```python
from build123d import *

# Parameters (mm, degrees)
SKETCH_1_W          = 58
SKETCH_1_H          = 62
EXTRUDE_1_DEPTH     = 10
SKETCH_2_W          = 46
SKETCH_2_H          = 62
CUT_EXTRUDE_1_DEPTH = 1.5
CHAMFER_1_SIZE      = 3
CUT_EXTRUDE_2_REACH = 45.293


with BuildPart() as part:
    # 草图1 → 凸台-拉伸1 (new body)
    with BuildSketch(Plane.XY):
        Rectangle(SKETCH_1_W, SKETCH_1_H)
    extrude(amount=EXTRUDE_1_DEPTH)

    # 草图2 → 切除-拉伸1 (cut)
    with BuildSketch(Plane.XY.offset(10)):
        Rectangle(SKETCH_2_W, SKETCH_2_H)
    extrude(amount=-CUT_EXTRUDE_1_DEPTH, mode=Mode.SUBTRACT)

    # 倒角1
    chamfer_1_edges = [part.edges().sort_by_distance(p)[0] for p in [
        (-29, 31, 5),
        (29, 31, 5),
    ]]
    chamfer(chamfer_1_edges, length=CHAMFER_1_SIZE)

    # 草图3 → 切除-拉伸2 (cut, up to next)
    with BuildSketch(Plane.XY.offset(8.5), mode=Mode.PRIVATE) as cut_extrude_2_sk1:
        with BuildLine():
            Line((-18.25, -24), (-18.25, -14))
            ThreePointArc((-18.25, -14), (-16, -11.75), (-13.75, -14))
            Line((-13.75, -14), (-13.75, -24))
            ThreePointArc((-13.75, -24), (-16, -26.25), (-18.25, -24))
        make_face()
    cut_extrude_2_tool1 = extrude(cut_extrude_2_sk1.sketch, amount=-CUT_EXTRUDE_2_REACH, mode=Mode.PRIVATE) & part.part
    cut_extrude_2 = cut_extrude_2_tool1.solids().sort_by_distance((-16, -19, 8.5))[0]
    add(cut_extrude_2, mode=Mode.SUBTRACT)

    # 镜向1: 切除-拉伸2 across plane
    add(cut_extrude_2.mirror(Plane(origin=(0, 0, 0), x_dir=(0, 0, 1), z_dir=(1, 0, 0))), mode=Mode.SUBTRACT)


solid = part.part
```
Verification items for the finished model (mm, model axes). A direction names the side the tool comes from. Round coordinates to 2 decimals unless told otherwise and drop trailing zeros. Loops run counter-clockwise (first coordinate to the right, second up) from the corner with the lowest first, then second, coordinate; pieces in that order, holes last. Notation, with made-up numbers: (36.25, 69.25) -> (49.25, 69.25) arc R26 ccw to (49.25, 102.25) -> close; hole circle Ø3 at (55.25, -24). An arc over 180 degrees is marked (long way). Answer as a JSON object with one key per item and string values.
Q1. Section check C-C (z = 3.5). Record the boundary of the cut face in (x, y).
Data:
{"outline": "(-29, -31) -> (29, -31) -> (29, 28) -> (26, 31) -> (-26, 31) -> (-29, 28) -> close; hole (-18.25, -24) arc R2.25 ccw to (-13.75, -24) -> (-13.75, -14) arc R2.25 ccw to (-18.25, -14) -> close; hole (13.75, -24) arc R2.25 ccw to (18.25, -24) -> (18.25, -14) arc R2.25 ccw to (13.75, -14) -> close"}
Q2. Section check B-B (x = 16). Record the boundary of the cut face in (y, z).
Data:
{"outline": "(-31, 0) -> (-26.25, 0) -> (-26.25, 8.5) -> (-31, 8.5) -> close; (-11.75, 0) -> (31, 0) -> (31, 8.5) -> (-11.75, 8.5) -> close"}
Q3. Section check A-A (y = -20). Record the boundary of the cut face in (x, z).
Data:
{"outline": "(-29, 0) -> (-18.25, 0) -> (-18.25, 8.5) -> (-23, 8.5) -> (-23, 10) -> (-29, 10) -> close; (-13.75, 0) -> (13.75, 0) -> (13.75, 8.5) -> (-13.75, 8.5) -> close; (18.25, 0) -> (29, 0) -> (29, 10) -> (23, 10) -> (23, 8.5) -> (18.25, 8.5) -> close"}
Q4. Go/stop test with a flat-tipped pin: P1, Ø10, axis at x = 15, y = 19.5, coming from the -Z side. Record where the tip stops, or that it passes through.
Data:
{"P1": "stops at z = 0"}
Q5. Section check D-D (z = 9.25). Record the boundary of the cut face in (x, y).
Data:
{"outline": "(-29, -31) -> (-23, -31) -> (-23, 31) -> (-26, 31) -> (-29, 28) -> close; (23, -31) -> (29, -31) -> (29, 28) -> (26, 31) -> (23, 31) -> close"}
Q6. Access from +Z, -Z, +X, -X, +Y, -Y to the whole of each face (thin tool, end or side, straight path). Record for faces 1 (the flat face through (-23, 0, 9)), 2 (the flat face through (-27, 30, 5)), 3 (the flat face through (13.75, -19, 4)).
Data:
{"face 1": "+Z, +Y, -Y", "face 2": "+Z, -Z, -X, +Y", "face 3": "+Z, -Z"}
Q7. Scan lines: line 1 (X direction, y = -23.5, z = 3.75); line 2 (X direction, y = -12, z = 6.5); line 3 (X direction, y = 13, z = 9.25). Record each from-to range of solid material in increasing order. Write a range as from..to.
Data:
{"line 1": "x = -29..-18.25, -13.75..13.75, 18.25..29", "line 2": "x = -29..-17.03, -14.97..14.97, 17.03..29", "line 3": "x = -29..-23, 23..29"}
Q8. Draft check along X on faces 4 (the flat face through (28, 29, 5)), 5 (the flat face through (0, 31, 5)), 6 (the flat face through (-13.75, -19, 4)). Enter one of: pulls with the +X half, pulls with the -X half, needs draft (parallel to the pull), parting line crosses it, or undercut.
Data:
{"face 4": "pulls with the +X half", "face 5": "needs draft", "face 6": "undercut"}
